```python
from build123d import *

# Parameters (mm, degrees)
SKETCH16_R     = 3.4
SKETCH16_R_2   = 3
MEMBER_1_DEPTH = 580


with BuildPart() as part:
    # Sketch16 → Member 1 (new body)
    with BuildSketch(Plane(origin=(0, 0, 0), x_dir=(-1, 0, 0), z_dir=(0, 1, 0))):
        with BuildLine():
            Line((-5.1, 20), (-5.1, 19.5))
            Line((-5.1, 19.5), (-4.1, 19.5))
            Line((-4.1, 19.5), (-4.1, 17))
            Line((-4.1, 17), (-6.1, 17))
            Line((-6.1, 17), (-6.1, 18))
            Line((-6.1, 18), (-10.3, 18))
            Line((-10.3, 18), (-10.3, 12))
            Line((-10.3, 12), (-6, 7.7))
            Line((-6, 7.7), (6, 7.7))
            Line((6, 7.7), (10.3, 12))
            Line((10.3, 12), (10.3, 18))
            Line((10.3, 18), (6.1, 18))
            Line((6.1, 18), (6.1, 17))
            Line((6.1, 17), (4.1, 17))
            Line((4.1, 17), (4.1, 19.5))
            Line((4.1, 19.5), (5.1, 19.5))
            Line((5.1, 19.5), (5.1, 20))
            Line((5.1, 20), (15.5, 20))
            ThreePointArc((15.5, 20), (18.681980515, 18.681980515), (20, 15.5))
            Line((20, 15.5), (20, 5.1))
            Line((20, 5.1), (19.5, 5.1))
            Line((19.5, 5.1), (19.5, 4.1))
            Line((19.5, 4.1), (17, 4.1))
            Line((17, 4.1), (17, 6.1))
            Line((17, 6.1), (18, 6.1))
            Line((18, 6.1), (18, 10.3))
            Line((18, 10.3), (12, 10.3))
            Line((12, 10.3), (7.7, 6))
            Line((7.7, 6), (7.7, -6))
            Line((7.7, -6), (12, -10.3))
            Line((12, -10.3), (18, -10.3))
            Line((18, -10.3), (18, -6.1))
            Line((18, -6.1), (17, -6.1))
            Line((17, -6.1), (17, -4.1))
            Line((17, -4.1), (19.5, -4.1))
            Line((19.5, -4.1), (19.5, -5.1))
            Line((19.5, -5.1), (20, -5.1))
            Line((20, -5.1), (20, -15.5))
            ThreePointArc((20, -15.5), (18.681980515, -18.681980515), (15.5, -20))
            Line((15.5, -20), (5.1, -20))
            Line((5.1, -20), (5.1, -19.5))
            Line((5.1, -19.5), (4.1, -19.5))
            Line((4.1, -19.5), (4.1, -17))
            Line((4.1, -17), (6.1, -17))
            Line((6.1, -17), (6.1, -18))
            Line((6.1, -18), (10.3, -18))
            Line((10.3, -18), (10.3, -12))
            Line((10.3, -12), (6, -7.7))
            Line((6, -7.7), (-6, -7.7))
            Line((-6, -7.7), (-10.3, -12))
            Line((-10.3, -12), (-10.3, -18))
            Line((-10.3, -18), (-6.1, -18))
            Line((-6.1, -18), (-6.1, -17))
            Line((-6.1, -17), (-4.1, -17))
            Line((-4.1, -17), (-4.1, -19.5))
            Line((-4.1, -19.5), (-5.1, -19.5))
            Line((-5.1, -19.5), (-5.1, -20))
            Line((-5.1, -20), (-15.5, -20))
            ThreePointArc((-15.5, -20), (-18.681980515, -18.681980515), (-20, -15.5))
            Line((-20, -15.5), (-20, -5.1))
            Line((-20, -5.1), (-19.5, -5.1))
            Line((-19.5, -5.1), (-19.5, -4.1))
            Line((-19.5, -4.1), (-17, -4.1))
            Line((-17, -4.1), (-17, -6.1))
            Line((-17, -6.1), (-18, -6.1))
            Line((-18, -6.1), (-18, -10.3))
            Line((-18, -10.3), (-12, -10.3))
            Line((-12, -10.3), (-7.7, -6))
            Line((-7.7, -6), (-7.7, 6))
            Line((-7.7, 6), (-12, 10.3))
            Line((-12, 10.3), (-18, 10.3))
            Line((-18, 10.3), (-18, 6.1))
            Line((-18, 6.1), (-17, 6.1))
            Line((-17, 6.1), (-17, 4.1))
            Line((-17, 4.1), (-19.5, 4.1))
            Line((-19.5, 4.1), (-19.5, 5.1))
            Line((-19.5, 5.1), (-20, 5.1))
            Line((-20, 5.1), (-20, 15.5))
            ThreePointArc((-20, 15.5), (-18.681980515, 18.681980515), (-15.5, 20))
            Line((-15.5, 20), (-5.1, 20))
        make_face()
        Circle(SKETCH16_R, mode=Mode.SUBTRACT)
        with Locations((-15.556349186, 15.556349186)):
            Circle(SKETCH16_R_2, mode=Mode.SUBTRACT)
        with Locations((15.556349186, 15.556349186)):
            Circle(SKETCH16_R_2, mode=Mode.SUBTRACT)
        with Locations((15.556349186, -15.556349186)):
            Circle(SKETCH16_R_2, mode=Mode.SUBTRACT)
        with Locations((-15.556349186, -15.556349186)):
            Circle(SKETCH16_R_2, mode=Mode.SUBTRACT)
    extrude(amount=MEMBER_1_DEPTH)


solid = part.part
```
Geometry: final body of the model. Coordinates: model frame, mm. A direction names the side the tool comes from. Coordinates: 2 decimals unless noted, no trailing zeros. Write each question's results on one line, items separated by ' | '.
1) Line query: line 1 (Z direction, x = 16, y = 107.5); line 2 (Z direction, x = 5.5, y = 260.5); line 3 (Z direction, x = 5, y = 497.5). Output: solid intervals per line, ascending. Write a range as from..to.
Results list:
line 1: -19.97..-18.52, -12.59..-10.3, 10.3..12.59, 18.52..19.97 | line 2: -20..-17, -7.7..7.7, 17..20 | line 3: -19.5..-17, -7.7..7.7, 17..19.5
2) Set-up query: faces 1 (the flat face through (-10, 286, -20)), 2 (the flat face through (7.7, 286, 0)). Return all of +Z, -Z, +X, -X, +Y, -Y with unobstructed straight access to the full face (end or side cutting, diameter ignored); none if empty.
Results list:
face 1: -Z, +X, -X, +Y, -Y | face 2: +Y, -Y
3) Pin query (flat end, axial travel): pin 1 (0.8 mm diameter, centred on y = 187, z = 17.5, fed in from -X); pin 2 (0.8 mm diameter, centred on x = 4.5, y = 428, fed in from +Z); pin 3 (2 mm diameter, centred on x = -17.5, y = 396.5, fed in from +Z). Return the tip coordinate at first contact, or that it passes through.
Results list:
pin 1: x = -19.71 | pin 2: z = 19.5 | pin 3: z = 19.89
4) Section A-A, the plane y = 441.5. State how many separate pieces and enclosed holes the cut face has, plus the area to 3 significant figures.
Results list:
separate pieces: 1 | enclosed holes: 5 | area: 605 mm^2
5) Pull-direction query (X, two-part tool) for faces 3 (the flat face through (-20, 286, -10)), 4 (the flat face through (20, 286, -10)), 5 (the flat face through (-7.7, 286, 0)); classes: pulls with the +X half, pulls with the -X half, needs draft (parallel to the pull), parting line crosses it, or undercut.
Results list:
face 3: pulls with the -X half | face 4: pulls with the +X half | face 5: undercut
